Verification items for the finished model (mm, model axes). Give positions to 0.01 mm unless a question says otherwise; leave off trailing zeros. Loops run counter-clockwise (first coordinate to the right, second up) from the corner with the lowest first, then second, coordinate; pieces in that order, holes last. Notation, with made-up numbers: (-26.75, 80) - (25.25, 80) arc R28 ccw to (25.25, 109) - close; hole circle Ø3 at (83, 15.5). An arc over 180 degrees is marked (long way). Answer in a Markdown table with one row per item.
```python
from build123d import *

# Parameters (mm, degrees)
BOSS_EXTRUDE1_DEPTH = 20


with BuildPart() as part:
    # Sketch1 → Boss-Extrude1 (new body)
    with BuildSketch(Plane.XY):
        Polygon((15783.129958129, 4624.359704887), (15687.257317346, 4624.359704887), (15446.728394371, 4424.359704449), (15446.728394371, 4374.359704887), (15783.129958129, 4374.359704887), (15783.129958129, 4384.359705726), (15863.129958392, 4400.769556521), (15863.129958392, 4597.949855679), (15783.129958129, 4614.359706473), align=None)
    extrude(amount=BOSS_EXTRUDE1_DEPTH)


solid = part.part
```
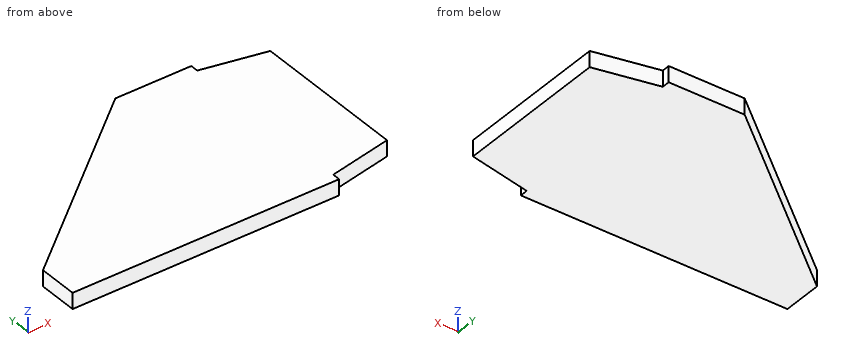
Q1. Sectioned sample at B-B (x = 15517.5). Record the cut outline in (y, z), and give its area (3 significant figures).
Completed:
| item | result |
|---|---|
| outline | (4374.36, 0) - (4483.21, 0) - (4483.21, 20) - (4374.36, 20) - close |
| area | 2,180 mm^2 |
Q2. Sectioned sample at C-C (y = 4530). Record the cut outline in (x, z).
Completed:
| item | result |
|---|---|
| outline | (15573.78, 0) - (15863.13, 0) - (15863.13, 20) - (15573.78, 20) - close |
Q3. Go/stop test with flat-tipped pins: P1, Ø5, axis at y = 4619, z = 11.5, coming from the +X side; P2, Ø10, axis at y = 4524, z = 4.5, coming from the -X side; P3, Ø5, axis at x = 15560.5, z = 3, coming from the +Y side. Record where each tip stops, or that it passes through.
Completed:
| item | result |
|---|---|
| P1 | x = 15783.13 |
| P2 | x = 15560.55 |
| P3 | y = 4521.04 |
Q4. Sectioned sample at A-A (z = 5.5). Record the cut outline in (x, y).
Completed:
| item | result |
|---|---|
| outline | (15446.73, 4374.36) - (15783.13, 4374.36) - (15783.13, 4384.36) - (15863.13, 4400.77) - (15863.13, 4597.95) - (15783.13, 4614.36) - (15783.13, 4624.36) - (15687.26, 4624.36) - (15446.73, 4424.36) - close |
Q5. Thickness scan on line 1 (X direction, y = 4492.5, z = 17); line 2 (Y direction, x = 15585.5, z = 10); line 3 (Y direction, x = 15633, z = 9.25). Record the ranges inside material, lowest first.
Completed:
| item | result |
|---|---|
| line 1 | 15528.68 to 15863.13 |
| line 2 | 4374.36 to 4539.75 |
| line 3 | 4374.36 to 4579.24 |
